Geometry: final body of the model. Coordinates: model frame, mm. Give positions to 0.01 mm unless a question says otherwise; leave off trailing zeros. Loops run counter-clockwise (first coordinate to the right, second up) from the corner with the lowest first, then second, coordinate; pieces in that order, holes last.
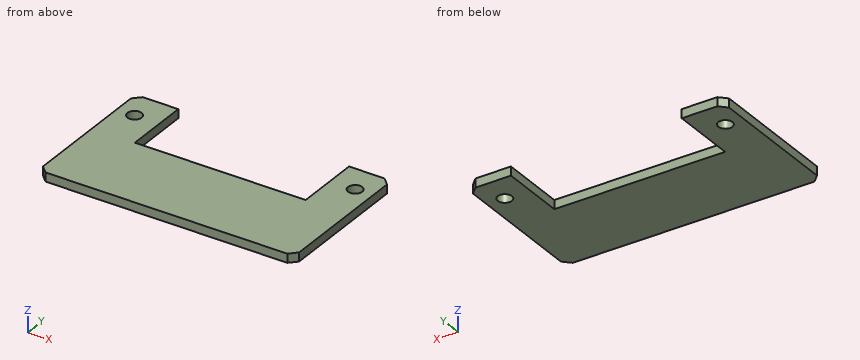
```python
from build123d import *

# Parameters (mm, degrees)
SKETCH1_R           = 20
BOSS_EXTRUDE1_DEPTH = 25
CHAMFER1_SIZE       = 20


with BuildPart() as part:
    # Sketch1 → Boss-Extrude1 (new body)
    with BuildSketch(Plane.XY):
        Polygon((120, 0), (0, 0), (0, -415), (720, -415), (720, 0), (600, 0), (600, -185), (120, -185), align=None)
        with Locations((50, -80)):
            Circle(SKETCH1_R, mode=Mode.SUBTRACT)
        with Locations((670, -80)):
            Circle(SKETCH1_R, mode=Mode.SUBTRACT)
    extrude(amount=BOSS_EXTRUDE1_DEPTH)

    # Chamfer1
    chamfer1_edges = [part.edges().sort_by_distance(p)[0] for p in [
        (720, 0, 12.5),
        (720, -415, 12.5),
        (0, -415, 12.5),
        (0, 0, 12.5),
    ]]
    chamfer(chamfer1_edges, length=CHAMFER1_SIZE)


solid = part.part
```
Q1. Section query C-C, the plane y = -80. Return loops of the section in (x, z), and give its area (3 significant figures).
Q2. Pin query (flat end, axial travel): pin 1 Ø4 at (x, z) = (131.5, 21) entering from +Y; pin 2 Ø24 at (x, y) = (50, -80) entering from +Z. Return the tip coordinate at first contact, or that it passes through.
Q3. Material intervals for probe 1 along X at (y, z) = (-82.5, 6); probe 2 along X at (y, z) = (-138.5, 11.5); probe 3 along Y at (x, z) = (50, 15.5), sorted ascending.
Q4. Section query D-D, the plane x = 331. Return loops of the section in (y, z).
Q5. Section query A-A, the plane x = 50. Return loops of the section in (y, z).
Q6. Section query B-B, the plane z = 12.25. Return loops of the section in (x, y), and give its area (3 significant figures).
Resolved:
1. outline: (0, 0) - (30, 0) - (30, 25) - (0, 25) - close; (70, 0) - (120, 0) - (120, 25) - (70, 25) - close; (600, 0) - (650, 0) - (650, 25) - (600, 25) - close; (690, 0) - (720, 0) - (720, 25) - (690, 25) - close
1. area: 4,000 mm2
2. pin 1: stops at y = -185
2. pin 2: passes through
3. probe 1: x = 0 to 30.16, 69.84 to 120, 600 to 650.16, 689.84 to 720
3. probe 2: x = 0 to 120, 600 to 720
3. probe 3: y = -415 to -100, -60 to 0
4. outline: (-415, 0) - (-185, 0) - (-185, 25) - (-415, 25) - close
5. outline: (-415, 0) - (-100, 0) - (-100, 25) - (-415, 25) - close; (-60, 0) - (0, 0) - (0, 25) - (-60, 25) - close
6. outline: (0, -395) - (20, -415) - (700, -415) - (720, -395) - (720, -20) - (700, 0) - (600, 0) - (600, -185) - (120, -185) - (120, 0) - (20, 0) - (0, -20) - close; hole circle Ø40 at (50, -80); hole circle Ø40 at (670, -80)
6. area: 207,000 mm2
